from build123d import *

# Parameters (mm, degrees)
SKETCH2_W               = 80
SKETCH2_H               = 140
BOSS_EXTRUDE1_DEPTH     = 30
CHAMFER1_SIZE           = 20
CUT_EXTRUDE1_DEPTH      = 111.453610172
CUT_EXTRUDE1_DEPTH_BACK = 111.453610172
SKETCH3_W               = 32
SKETCH3_H               = 180
FILLET1_R               = 5
CUT_EXTRUDE2_DEPTH      = 101.498756211
CUT_EXTRUDE2_DEPTH_BACK = 101.498756211
SKETCH4_R               = 20
CHAMFER2_SIZE           = 1.5
M24_TAPPED_HOLE1_D      = 21


with BuildPart() as part:
    # Sketch2 → Boss-Extrude1 (new, symmetric)
    with BuildSketch(Plane.XY):
        Rectangle(SKETCH2_W, SKETCH2_H)
    extrude(amount=BOSS_EXTRUDE1_DEPTH, both=True)

    # Chamfer1
    chamfer1_edges = [part.edges().sort_by_distance(p)[0] for p in [
        (-40, 70, 0),
        (40, 70, 0),
    ]]
    chamfer(chamfer1_edges, length=CHAMFER1_SIZE)

    # Sketch3 → Cut-Extrude1 (cut, two sides: drawn at the far end of the back side and taken through both)
    with BuildSketch(Plane.ZY.offset(40).offset(-CUT_EXTRUDE1_DEPTH_BACK)):
        with Locations((0, 70)):
            Rectangle(SKETCH3_W, SKETCH3_H)
    extrude(amount=CUT_EXTRUDE1_DEPTH + CUT_EXTRUDE1_DEPTH_BACK, mode=Mode.SUBTRACT)

    # Fillet1
    fillet1_edges = [part.edges().sort_by_distance(p)[0] for p in [
        (0, -20, 16),
        (0, -20, -16),
    ]]
    fillet(fillet1_edges, radius=FILLET1_R)

    # Sketch4 → Cut-Extrude2 (cut, two sides: drawn at the far end of the back side and taken through both)
    with BuildSketch(Plane.XY.offset(30).offset(-CUT_EXTRUDE2_DEPTH_BACK)):
        with Locations((0, 35)):
            Circle(SKETCH4_R)
    extrude(amount=CUT_EXTRUDE2_DEPTH + CUT_EXTRUDE2_DEPTH_BACK, mode=Mode.SUBTRACT)

    # Chamfer2
    chamfer2_edges = [part.edges().sort_by_distance(p)[0] for p in [
        (-20, 35, 30),
        (-20, 35, -30),
    ]]
    chamfer(chamfer2_edges, length=CHAMFER2_SIZE)

    # M24 Tapped Hole1 (through all)
    with Locations(Plane(origin=(0, -20, 0), x_dir=(1, 0, 0), z_dir=(0, 1, 0))):
        with Locations((0, 0)):
            Hole(M24_TAPPED_HOLE1_D / 2)


solid = part.part
Geometry: final body of the model. Coordinates: model frame, mm. A direction names the side the tool comes from. Round coordinates to 2 decimals unless told otherwise and drop trailing zeros. Order: outer loops, then holes, each group sorted by start corner. A loop starts at its lowest first (then second) coordinate and runs counter-clockwise, first axis right, second up. Notation, with made-up numbers: (6, -16) -> (32, -16) arc R29 cw to (32, 19) -> close; hole circle Ø1 at (-32.75, -15). An arc over 180 degrees is marked (long way). Put each result on its own line as item: value. Start each with the question number.
Q1. Line query: probe 1 along Z at (x, y) = (0, -54.5); probe 2 along X at (y, z) = (35, 21.5); probe 3 along Y at (x, z) = (0, -23.5). Output: solid intervals per line, ascending.
Q2. Section D-D on y = 6. Return the cut outline in (x, z).
Q3. Pull-direction query (Y, two-part tool) for faces 3 (the cylindrical face through (-1, -19, -14)), 4 (the cylindrical face through (-2.6, 54.83, -22.34)), 5 (the flat face through (-9, -70, 7)), 6 (the cylindrical face through (-2.6, 54.83, 22.16)); classes: +Y half, -Y half, draft (parallel to the pull), parting line (faces both ways), or undercut.
Q4. Section B-B on x = 0. Return the cut outline in (y, z), and give its area (3 significant figures).
Q5. Section C-C on z = 0. Return the cut outline in (x, y).
Q6. First-contact query: pin 1 (6.5 mm diameter, centred on x = 14.5, z = 3, fed in from +Y); pin 2 (5 mm diameter, centred on x = 28.5, z = 20, fed in from +Y). Flat tips, straight axial feed; report the tip coordinate or a pass-through.
Q7. Reachability of faces 1 (the cylindrical face through (-1, -18, 15)), 2 (the flat face through (-1, -15, 30)) from +Z, -Z, +X, -X, +Y, -Y: full face, straight path, thin tool, end or side. Return the list, or none.
Q8. Section A-A on y = 35. Return the cut outline in (x, z).
Ans:
1. probe 1: z = -30 to -10.5, 10.5 to 30
1. probe 2: x = -40 to -20, 20 to 40
1. probe 3: y = -70 to 15, 55 to 70
2. outline: (-40, -30) -> (40, -30) -> (40, -16) -> (-40, -16) -> close; (-40, 16) -> (40, 16) -> (40, 30) -> (-40, 30) -> close
3. face 3: +Y half
3. face 4: undercut
3. face 5: -Y half
3. face 6: undercut
4. outline: (-70, -30) -> (13.5, -30) -> (15, -28.5) -> (15, -16) -> (-15, -16) arc R5 cw to (-20, -11) -> (-20, -10.5) -> (-70, -10.5) -> close; (-70, 10.5) -> (-20, 10.5) -> (-20, 11) arc R5 cw to (-15, 16) -> (15, 16) -> (15, 28.5) -> (13.5, 30) -> (-70, 30) -> close; (55, -28.5) -> (56.5, -30) -> (70, -30) -> (70, -16) -> (55, -16) -> close; (55, 16) -> (70, 16) -> (70, 30) -> (56.5, 30) -> (55, 28.5) -> close
4. area: 3,360 mm2
5. outline: (-40, -70) -> (-10.5, -70) -> (-10.5, -20) -> (-40, -20) -> close; (10.5, -70) -> (40, -70) -> (40, -20) -> (10.5, -20) -> close
6. pin 1: stops at y = -20
6. pin 2: stops at y = 64
7. face 1: +X, -X, +Y
7. face 2: +Z, +X, -X, +Y, -Y
8. outline: (-40, -30) -> (-21.5, -30) -> (-20, -28.5) -> (-20, -16) -> (-40, -16) -> close; (-40, 16) -> (-20, 16) -> (-20, 28.5) -> (-21.5, 30) -> (-40, 30) -> close; (20, -28.5) -> (21.5, -30) -> (40, -30) -> (40, -16) -> (20, -16) -> close; (20, 16) -> (40, 16) -> (40, 30) -> (21.5, 30) -> (20, 28.5) -> close
